Can you work these out from the drawing? Everything is in mm from the part's minimum corner. Give positions to 0.01 mm unless a question says otherwise; leave off trailing zeros. Write each loop counter-clockwise with the first axis right and the second up, starting at its lowest first coordinate (ties: lowest second). Pieces come first, ordered by that corner, then holes. Notation, with made-up numbers: (42, -39) -> (96, -39) arc R26 ccw to (96, -9) -> close; hole circle Ø1 at (72.5, 25). An arc over 180 degrees is marked (long way). Return JSON: item names as keys, results as strings.
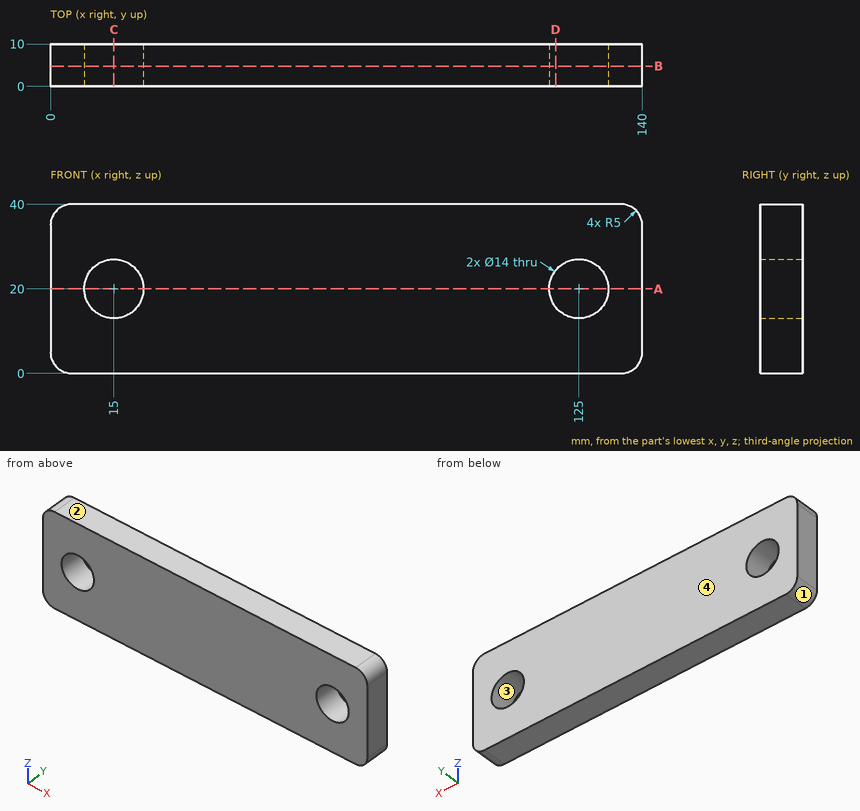
1. If we mould it in two halves opening along Z, with no side actions, what happens to the marked faces 1, 2, 3 and 4? For each: released by +Z, released by -Z, zero draft, split by the parting line, or undercut.
Taken from the geometry:
{"face 1": "released by -Z", "face 2": "released by +Z", "face 3": "undercut", "face 4": "zero draft"}
2. Suppose I cut it at C-C, the plane x = 15. List the corners of the cut face in (y, z) for me, and give its area (3 significant figures).
Taken from the geometry:
{"outline": "(0, 0) -> (10, 0) -> (10, 13) -> (0, 13) -> close; (0, 27) -> (10, 27) -> (10, 40) -> (0, 40) -> close", "area": "260 mm²"}
3. Suppose I cut it at A-A, the plane z = 20. List the corners of the cut face in (x, y) for me.
Taken from the geometry:
{"outline": "(0, 0) -> (8, 0) -> (8, 10) -> (0, 10) -> close; (22, 0) -> (118, 0) -> (118, 10) -> (22, 10) -> close; (132, 0) -> (140, 0) -> (140, 10) -> (132, 10) -> close"}
4. Suppose I cut it at B-B, the plane y = 4.75. List the corners of the cut face in (x, z) for me.
Taken from the geometry:
{"outline": "(0, 5) arc R5 ccw to (5, 0) -> (135, 0) arc R5 ccw to (140, 5) -> (140, 35) arc R5 ccw to (135, 40) -> (5, 40) arc R5 ccw to (0, 35) -> close; hole circle Ø14 at (15, 20); hole circle Ø14 at (125, 20)"}
5. Suppose I cut it at D-D, the plane x = 119.5. List the corners of the cut face in (y, z) for me, and give its area (3 significant figures).
Taken from the geometry:
{"outline": "(0, 0) -> (10, 0) -> (10, 15.67) -> (0, 15.67) -> close; (0, 24.33) -> (10, 24.33) -> (10, 40) -> (0, 40) -> close", "area": "313 mm²"}
6. If I drill on line 1 (X direction, y = 7.75, z = 20); line 2 (Z direction, x = 125, y = 7.25); line 3 (X direction, y = 1, z = 26), over which ranges is the centre line in solid material (lowest first)? Write a range as [from, to].
Taken from the geometry:
{"line 1": "x = [0, 8], [22, 118], [132, 140]", "line 2": "z = [0, 13], [27, 40]", "line 3": "x = [0, 11.39], [18.61, 121.39], [128.61, 140]"}
7. For pin 1 Ø4 at (x, z) = (47.5, 13.5) entering from -Y; pin 2 Ø8.5 at (x, z) = (15, 20) entering from -Y, each with a flat end and sliding along its axis, tell me the tip position at first contact or that it passes through.
Taken from the geometry:
{"pin 1": "stops at y = 0", "pin 2": "passes through"}
